from build123d import *

# Parameters (mm, degrees)
SKETCH_1_W          = 22
SKETCH_1_H          = 56
EXTRUDE_1_DEPTH     = 8
CUT_EXTRUDE_1_DEPTH = 3
SKETCH_9_R          = 3
EXTRUDE_2_DEPTH     = 87
SKETCH_10_R         = 3
EXTRUDE_3_DEPTH     = 87
SKETCH_11_R         = 3
EXTRUDE_4_DEPTH     = 59.5
SKETCH_12_R         = 6
EXTRUDE_5_DEPTH     = 5


with BuildPart() as part:
    # 草图1 → 凸台-拉伸1 (new body)
    with BuildSketch(Plane.XY):
        Rectangle(SKETCH_1_W, SKETCH_1_H)
    extrude(amount=-EXTRUDE_1_DEPTH)

    # 草图2 → 切除-旋转1 (revolve, cut)
    with BuildSketch(Plane(origin=(0, 24, 0), x_dir=(1, 0, 0), z_dir=(0, 1, 0)), mode=Mode.PRIVATE) as cut_revolve_1_sk:
        Polygon((-7, 0), (-9, 0), (-8.621, 0.379), (-8.621, 7.621), (-9, 8), (-7, 8), align=None)
    revolve(cut_revolve_1_sk.sketch.rotate(Axis((-7, 24, -8), (0, 0, 1)), 180), axis=Axis((-7, 24, -8), (0, 0, 1)), mode=Mode.SUBTRACT)

    # 草图3 → 切除-旋转2 (revolve, cut)
    with BuildSketch(Plane(origin=(0, -24, 0), x_dir=(1, 0, 0), z_dir=(0, 1, 0)), mode=Mode.PRIVATE) as cut_revolve_2_sk:
        Polygon((-7, 0), (-9, 0), (-8.621, 0.379), (-8.621, 7.621), (-9, 8), (-7, 8), align=None)
    revolve(cut_revolve_2_sk.sketch.rotate(Axis((-7, -24, -8), (0, 0, 1)), 180), axis=Axis((-7, -24, -8), (0, 0, 1)), mode=Mode.SUBTRACT)

    # 草图4 → 切除-旋转3 (revolve, cut)
    with BuildSketch(Plane(origin=(0, -24, 0), x_dir=(1, 0, 0), z_dir=(0, 1, 0)), mode=Mode.PRIVATE) as cut_revolve_3_sk:
        Polygon((7, 0), (5, 0), (5.379, 0.379), (5.379, 7.621), (5, 8), (7, 8), align=None)
    revolve(cut_revolve_3_sk.sketch.rotate(Axis((7, -24, -8), (0, 0, 1)), 180), axis=Axis((7, -24, -8), (0, 0, 1)), mode=Mode.SUBTRACT)

    # 草图5 → 切除-旋转4 (revolve, cut)
    with BuildSketch(Plane(origin=(0, 24, 0), x_dir=(1, 0, 0), z_dir=(0, 1, 0)), mode=Mode.PRIVATE) as cut_revolve_4_sk:
        Polygon((7, 0), (5, 0), (5.379, 0.379), (5.379, 7.621), (5, 8), (7, 8), align=None)
    revolve(cut_revolve_4_sk.sketch.rotate(Axis((7, 24, -8), (0, 0, 1)), 180), axis=Axis((7, 24, -8), (0, 0, 1)), mode=Mode.SUBTRACT)

    # 草图6 → 切除-旋转5 (revolve, cut)
    with BuildSketch(Plane(origin=(0, 0, 0), x_dir=(0, 0, -1), z_dir=(1, 0, 0)), mode=Mode.PRIVATE) as cut_revolve_5_sk:
        Polygon((0, 11.5), (0, 13), (6, 13), (6.866025404, 11.5), align=None)
    revolve(cut_revolve_5_sk.sketch.rotate(Axis((0, 11.5, -6.866025404), (0, 0, 1)), 270), axis=Axis((0, 11.5, -6.866025404), (0, 0, 1)), mode=Mode.SUBTRACT)

    # 草图7 → 切除-旋转6 (revolve, cut)
    with BuildSketch(Plane(origin=(0, 0, 0), x_dir=(0, 0, -1), z_dir=(1, 0, 0)), mode=Mode.PRIVATE) as cut_revolve_6_sk:
        Polygon((0, -11.5), (0, -10), (6, -10), (6.866025404, -11.5), align=None)
    revolve(cut_revolve_6_sk.sketch.rotate(Axis((0, -11.5, -6.866025404), (0, 0, 1)), 270), axis=Axis((0, -11.5, -6.866025404), (0, 0, 1)), mode=Mode.SUBTRACT)

    # 草图8 → 切除-拉伸1 (cut)
    with BuildSketch(Plane.XY):
        with BuildLine():
            Line((1.5, 11.25), (1.5, 11.75))
            ThreePointArc((1.5, 11.75), (0, 13.25), (-1.5, 11.75))
            Line((-1.5, 11.75), (-1.5, 11.25))
            ThreePointArc((-1.5, 11.25), (0, 9.75), (1.5, 11.25))
        make_face()
    extrude(amount=-CUT_EXTRUDE_1_DEPTH, mode=Mode.SUBTRACT)

    # 草图9 → 凸台-拉伸2 (add)
    with BuildSketch(Plane.XY.offset(-8)):
        with Locations((0, 20.5)):
            Circle(SKETCH_9_R)
    extrude(amount=-EXTRUDE_2_DEPTH)

    # 草图10 → 凸台-拉伸3 (add)
    with BuildSketch(Plane.XY.offset(-8)):
        with Locations((0, -20.5)):
            Circle(SKETCH_10_R)
    extrude(amount=-EXTRUDE_3_DEPTH)

    # 草图11 → 凸台-拉伸4 (add)
    with BuildSketch(Plane.XY.offset(-8)):
        Circle(SKETCH_11_R)
    extrude(amount=-EXTRUDE_4_DEPTH)

    # 草图12 → 凸台-拉伸5 (add)
    with BuildSketch(Plane.XY.offset(-70)):
        Circle(SKETCH_12_R)
    extrude(amount=EXTRUDE_5_DEPTH)


solid = part.part
Check sheet for the modelled part. Datum: model origin and axes. Units: mm. A direction names the side the tool comes from. Give positions to 0.01 mm unless a question says otherwise; leave off trailing zeros. Loops run counter-clockwise (first coordinate to the right, second up) from the corner with the lowest first, then second, coordinate; pieces in that order, holes last. Notation, with made-up numbers: M 75.5,-2 L 101.5,-2 A14 ccw 101.5,2 Z; hole C 35.5,14.25 d11. An arc over 180 degrees is marked long. Answer as a JSON object with one key per item and string values. Group by question number.
Q1. Access from +Z, -Z, +X, -X, +Y, -Y to the whole of each face (thin tool, end or side, straight path). Record for faces 4 (the flat face through (-3, -1, -65)), 5 (the cylindrical face through (-0.65, -23.43, -50.89)), 6 (the flat face through (0, 0, -70)), 7 (the cylindrical face through (0.03, 13.25, -1.48)).
Q2. Release check for a two-part mould opening along X. For faces 1 (the flat face through (11, 0, -4)), 2 (the cylindrical face through (5.714, 23.014, -4.051)), 3 (the flat face through (0, 28, -4)) record: released by +X, released by -X, zero draft, split by the parting line, or undercut.
Q3. Material ranges on line 1 along Y through (x, z) = (7, -5.5); line 2 along Y through (x, z) = (0, -2.3); line 3 along Z through (x, y) = (5.25, -0.5), recorded low to high. Write a range as [from, to].
Q4. Cross-section at B-B on z = -76. Record the cut outline in (x, y), then the cut area to 3 significant figures.
Q5. Cross-section at A-A on y = 0. Record the cut outline in (x, z), then the cut area to 3 significant figures.
Q6. Cross-section at C-C on z = -29. Record the cut outline in (x, y), then the cut area to 3 significant figures.
Q7. Go/stop test with flat-tipped pins: P1, Ø6, axis at x = -2, z = -39, coming from the +Y side; P2, Ø6, axis at x = 0.5, y = -1, coming from the -Z side; P3, Ø0.9, axis at x = -0.5, y = 10.5, coming from the +Z side. Record where each tip stops, or that it passes through.
Q8. Cross-section at D-D on y = -20.5. Record the cut outline in (x, z).
Evaluation:
{
 "1": {"face 4": "none", "face 5": "-Z", "face 6": "-Z, +X, -X", "face 7": "+Z"},
 "2": {"face 1": "released by +X", "face 2": "undercut", "face 3": "zero draft"},
 "3": {"line 1": "y = [-28, -25.62], [-22.38, 22.38], [25.62, 28]", "line 2": "y = [-28, -13], [-10, 9.75], [13.25, 28]", "line 3": "z = [-70, -65], [-8, 0]"},
 "4": {"outline": "C 0,-20.5 d6; C 0,20.5 d6", "area": "56.5 mm2"},
 "5": {"outline": "M -11,-8 L -3,-8 L -3,-65 L -6,-65 L -6,-70 L 6,-70 L 6,-65 L 3,-65 L 3,-8 L 11,-8 L 11,0 L -11,0 Z", "area": "578 mm2"},
 "6": {"outline": "C 0,-20.5 d6; C 0,0 d6; C 0,20.5 d6", "area": "84.8 mm2"},
 "7": {"P1": "stops at y = 23.5", "P2": "stops at z = -70", "P3": "stops at z = -3"},
 "8": {"outline": "M -11,-8 L -3,-8 L -3,-95 L 3,-95 L 3,-8 L 11,-8 L 11,0 L -11,0 Z"}
}
